Could you check a few things on this model? Use its own coordinates, in mm. A direction names the side the tool comes from. Give positions to 0.01 mm unless a question says otherwise; leave off trailing zeros. Order: outer loops, then holes, each group sorted by start corner. A loop starts at its lowest first (then second) coordinate and runs counter-clockwise, first axis right, second up.
from build123d import *

# Parameters (mm, degrees)
BOSS_EXTRUDE3_DEPTH                    = 45
CBORE_FOR_M5_HEX_CAP_SCREW1_AT_2_COUNT = 2
CBORE_FOR_M5_HEX_CAP_SCREW1_AT_2_PITCH = 120
CUT_EXTRUDE1_DEPTH                     = 10
SKETCH13_R                             = 15
CUT_EXTRUDE2_DEPTH                     = 2
SKETCH14_R                             = 1.204328259
SKETCH14_R_2                           = 1.2
CUT_EXTRUDE3_DEPTH                     = 5


with BuildPart() as part:
    # Sketch7 → Boss-Extrude3 (new body)
    with BuildSketch(Plane(origin=(0, 0, 0), x_dir=(1, 0, 0), z_dir=(0, 1, 0))):
        Polygon((0, 0), (55, 0), (55, 50), (115, 50), (115, 0), (170, 0), (170, 5), (120, 5), (120, 55), (50, 55), (50, 5), (0, 5), align=None)
    extrude(amount=BOSS_EXTRUDE3_DEPTH)

    # Sketch10 → CBORE for M5 Hex Cap Screw1 (revolve, cut)
    with BuildSketch(Plane(origin=(145, 22.5, -5), x_dir=(0, 1, 0), z_dir=(1, 0, 0))):
        Polygon((0, 0), (0, 5), (2.75, 5), (2.75, 3.5), (6.119, 3.5), (6.119, 0.025), (6.144, 0), align=None)
    cbore_for_m5_hex_cap_screw1 = revolve(axis=Axis((145, 22.5, -11.35), (0, 0, 1)), mode=Mode.SUBTRACT)

    # CBORE for M5 Hex Cap Screw1 at 2: CBORE for M5 Hex Cap Screw1 ×2
    with Locations(*[(-i * CBORE_FOR_M5_HEX_CAP_SCREW1_AT_2_PITCH, 0, 0) for i in range(1, CBORE_FOR_M5_HEX_CAP_SCREW1_AT_2_COUNT)]):
        add(cbore_for_m5_hex_cap_screw1, mode=Mode.SUBTRACT)

    # Sketch12 → Cut-Extrude1 (cut)
    with BuildSketch(Plane(origin=(0, 0, -55), x_dir=(-1, 0, 0), z_dir=(0, 0, -1))):
        with BuildLine():
            ThreePointArc((-77, 22.5), (-82.745606781, 30.175787335), (-91.729427803, 26.826060731))
            Line((-91.729427803, 26.826060731), (-78.270572197, 18.173939269))
            ThreePointArc((-78.270572197, 18.173939269), (-77.324212665, 20.245606781), (-77, 22.5))
        make_face()
        with BuildLine():
            Line((-78.270572197, 18.173939269), (-91.729427803, 26.826060731))
            ThreePointArc((-91.729427803, 26.826060731), (-89.326060731, 15.770572197), (-78.270572197, 18.173939269))
        make_face()
    extrude(amount=-CUT_EXTRUDE1_DEPTH, mode=Mode.SUBTRACT)

    # Sketch13 → Cut-Extrude2 (cut)
    with BuildSketch(Plane(origin=(0, 0, -55), x_dir=(-1, 0, 0), z_dir=(0, 0, -1))):
        with Locations((-85, 22.5)):
            Circle(SKETCH13_R)
    extrude(amount=-CUT_EXTRUDE2_DEPTH, mode=Mode.SUBTRACT)

    # Sketch14 → Cut-Extrude3 (cut)
    with BuildSketch(Plane(origin=(0, 0, -55), x_dir=(-1, 0, 0), z_dir=(0, 0, -1))):
        with Locations((-60, 5)):
            Circle(SKETCH14_R)
        with Locations((-60, 40)):
            Circle(SKETCH14_R_2)
        with Locations((-110, 5)):
            Circle(SKETCH14_R_2)
        with Locations((-110, 40)):
            Circle(SKETCH14_R_2)
    extrude(amount=-CUT_EXTRUDE3_DEPTH, mode=Mode.SUBTRACT)


solid = part.part
Item 1: For faces 1 (the cylindrical face through (78.08, 9.19, -54.01)), 2 (the flat face through (115, 22, -25)), 3 (the flat face through (20, 17, -5)), which set-ups out of +Z, -Z, +X, -X, +Y, -Y let a thin tool reach every point of the face, with its end or its side?
Findings:
face 1: -Z
face 2: +Z, +Y, -Y
face 3: -Z, -X, +Y, -Y
Item 2: Imagine slicing it at A-A on x = 145. List the corners of the cut face in (y, z) for me (3 decimals), then the cut area to 3 significant figures.
Findings:
outline: (0, -5) - (16.356, -5) - (16.381, -4.975) - (16.381, -1.5) - (19.75, -1.5) - (19.75, 0) - (0, 0) - close; (25.25, -1.5) - (28.619, -1.5) - (28.619, -4.975) - (28.644, -5) - (45, -5) - (45, 0) - (25.25, 0) - close
area: 174 mm2
Item 3: Imagine slicing it at B-B on z = -29.5. List the corners of the cut face in (x, y) for me.
Findings:
outline: (50, 0) - (55, 0) - (55, 45) - (50, 45) - close; (115, 0) - (120, 0) - (120, 45) - (115, 45) - close
Item 4: Imagine slicing it at C-C on y = 11.5. List the corners of the cut face in (x, z) for me, then the cut area to 3 significant figures.
Findings:
outline: (0, -5) - (50, -5) - (50, -55) - (74.8, -55) - (74.8, -53) - (95.2, -53) - (95.2, -55) - (120, -55) - (120, -5) - (170, -5) - (170, 0) - (115, 0) - (115, -50) - (55, -50) - (55, 0) - (0, 0) - close
area: 1,310 mm2
Item 5: Please list where these lines run through material, in increasing order: line 1 along X through (y, z) = (22.5, -3.55); line 2 along X through (y, z) = (10, -11.5); line 3 along Y through (x, z) = (60, -51.6).
Findings:
line 1: x = 0 to 18.88, 31.12 to 55, 115 to 138.88, 151.12 to 170
line 2: x = 50 to 55, 115 to 120
line 3: y = 0 to 3.8, 6.2 to 38.8, 41.2 to 45
Item 6: We'd pull the mould along X, two halves only. Please class faces 4 (the flat face through (148, 21, -1.5)), 5 (the flat face through (170, 22, -2)), 6 (the flat face through (140, 17, -5)): +X half, -X half, draft (parallel to the pull), parting line (faces both ways), or undercut.
Findings:
face 4: undercut
face 5: +X half
face 6: draft
Item 7: For pin 1 (10 mm diameter, centred on x = 145.5, y = 23, fed in from -Z); pin 2 (22.5 mm diameter, centred on y = 21.5, z = -34, fed in from +X); pin 3 (16 mm diameter, centred on x = 25, y = 22.5, fed in from -Z); pin 4 (2 mm diameter, centred on x = 110, y = 40, fed in from -Z), each with a flat end and sliding along its axis, tell me the tip position at first contact or that it passes through.
Findings:
pin 1: stops at z = -1.5
pin 2: stops at x = 120
pin 3: stops at z = -5
pin 4: passes through
Item 8: Imagine slicing it at D-D on x = 47. List the corners of the cut face in (y, z) for me.
Findings:
outline: (0, -5) - (45, -5) - (45, 0) - (0, 0) - close
